Check sheet for the modelled part. Datum: model origin and axes. Units: mm. Round coordinates to 2 decimals unless told otherwise and drop trailing zeros. Loops run counter-clockwise (first coordinate to the right, second up) from the corner with the lowest first, then second, coordinate; pieces in that order, holes last. Notation, with made-up numbers: (-23.75, 7) - (-6.75, 7) arc R8 ccw to (-6.75, 13) - close; hole circle Ø1 at (-37.75, 68.25). An arc over 180 degrees is marked (long way). Put each result on its own line as item: value.
```python
from build123d import *

# Parameters (mm, degrees)
HANDLE_PROFILE_SKETCH_R        = 0.09375
HANDLE_BAR_EXTRUDE_DEPTH       = 0.125
SCALE_X25_4_TO_INCH_SIZE_SCALE = 25.4


with BuildPart() as part:
    # Handle Profile Sketch → Handle Bar Extrude (new, symmetric)
    with BuildSketch(Plane.XY):
        with BuildLine():
            Line((-2, 0.25), (2, 0.25))
            ThreePointArc((2, 0.25), (2.25, 0), (2, -0.25))
            Line((2, -0.25), (-2, -0.25))
            ThreePointArc((-2, -0.25), (-2.25, 0), (-2, 0.25))
        make_face()
        with Locations((2, 0)):
            Circle(HANDLE_PROFILE_SKETCH_R, mode=Mode.SUBTRACT)
        with Locations((1.5, 0)):
            Circle(HANDLE_PROFILE_SKETCH_R, mode=Mode.SUBTRACT)
    extrude(amount=HANDLE_BAR_EXTRUDE_DEPTH, both=True)


with BuildPart() as part_1:
    # Scale x25.4 to Inch Size: scaled about (0, 0, 0)
    add(part.part.scale(SCALE_X25_4_TO_INCH_SIZE_SCALE))


solid = part_1.part
```
Item 1: Section check D-D on y = -4.75. Enter the section's corners in (x, z) (3 decimals).
Filled sheet:
outline: (-55.014, -3.175) - (55.014, -3.175) - (55.014, 3.175) - (-55.014, 3.175) - close
Item 2: Go/stop test with flat-tipped pins: pin 1 (3 mm diameter, centred on y = -2.5, z = 0, fed in from -X); pin 2 (3 mm diameter, centred on y = -4, z = -1, fed in from +X); pin 3 (1.5 mm diameter, centred on y = -1, z = -2, fed in from +X). Record where each tip stops, or that it passes through.
Filled sheet:
pin 1: x = -57.07
pin 2: x = 56.64
pin 3: x = 57.15
Item 3: Section check A-A on x = 38.1. Enter the section's corners in (y, z) (3 decimals), then the cut area to 3 significant figures.
Filled sheet:
outline: (-6.35, -3.175) - (-2.381, -3.175) - (-2.381, 3.175) - (-6.35, 3.175) - close; (2.381, -3.175) - (6.35, -3.175) - (6.35, 3.175) - (2.381, 3.175) - close
area: 50.4 mm²
Item 4: Thickness scan on line 1 (Y direction, x = 50.8, z = 1); line 2 (X direction, y = -0.5, z = 0). Record the ranges inside material, lowest first. Write a range as from..to.
Filled sheet:
line 1: -6.35..-2.38, 2.38..6.35
line 2: -57.13..35.77, 40.43..48.47, 53.13..57.13
Item 5: Section check B-B on y = 0. Enter the section's corners in (x, z) (3 decimals).
Filled sheet:
outline: (-57.15, -3.175) - (35.719, -3.175) - (35.719, 3.175) - (-57.15, 3.175) - close; (40.481, -3.175) - (48.419, -3.175) - (48.419, 3.175) - (40.481, 3.175) - close; (53.181, -3.175) - (57.15, -3.175) - (57.15, 3.175) - (53.181, 3.175) - close
Item 6: Release check for a two-part mould opening along Y. For faces 1 (the flat face through (1, 0, -3.175)), 2 (the cylindrical face through (57.15, 0.14, 0.04)), 3 (the cylindrical face through (35.72, 0.1, -0.04)), 4 (the cylindrical face through (48.91, -1.45, -0.04)) record: +Y half, -Y half, draft (parallel to the pull), parting line (faces both ways), or undercut.
Filled sheet:
face 1: draft
face 2: parting line
face 3: undercut
face 4: undercut
Item 7: Section check C-C on z = 0. Enter the section's corners in (x, y).
Filled sheet:
outline: (-50.8, -6.35) - (50.8, -6.35) arc R6.35 ccw to (50.8, 6.35) - (-50.8, 6.35) arc R6.35 ccw to start; hole circle Ø4.76 at (38.1, 0); hole circle Ø4.76 at (50.8, 0)
